```python
from build123d import *

# Parameters (mm, degrees)
EXTRUDE_1_DEPTH     = 6
SKETCH_2_W          = 12
SKETCH_2_H          = 12
CUT_EXTRUDE_1_DEPTH = 20


with BuildPart() as part:
    # 草图1 → 凸台-拉伸1 (new body)
    with BuildSketch(Plane.XY):
        with BuildLine():
            Line((3, 0), (17, 0))
            ThreePointArc((17, 0), (19.121320344, 0.878679656), (20, 3))
            ThreePointArc((20, 3), (19.121320344, 5.121320344), (17, 6))
            Line((17, 6), (3, 6))
            ThreePointArc((3, 6), (0.878679656, 5.121320344), (0, 3))
            ThreePointArc((0, 3), (0.878679656, 0.878679656), (3, 0))
        make_face()
    extrude(amount=EXTRUDE_1_DEPTH)

    # 草图2 → 切除-拉伸1 (cut)
    with BuildSketch(Plane(origin=(0, 0, 0), x_dir=(0, 0, -1), z_dir=(1, 0, 0))):
        with Locations((-3, 3)):
            Rectangle(SKETCH_2_W, SKETCH_2_H)
        Polygon((-6, 5.7), (-6, 0.3), (-5.7, 0), (-0.3, 0), (0, 0.3), (0, 5.7), (-0.3, 6), (-5.7, 6), align=None, mode=Mode.SUBTRACT)
    extrude(amount=CUT_EXTRUDE_1_DEPTH, mode=Mode.SUBTRACT)


solid = part.part
```
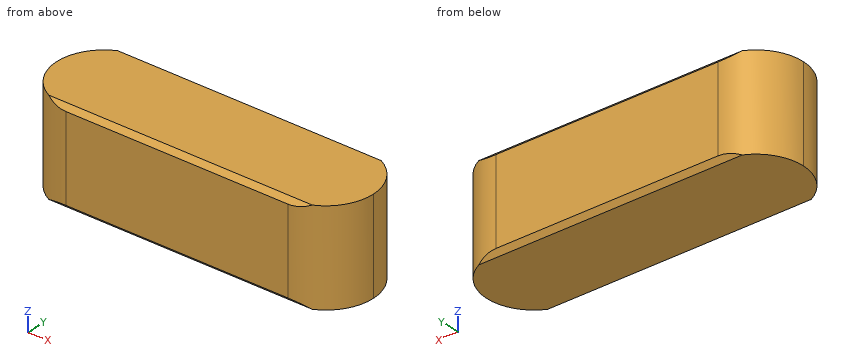
Geometry: final body of the model. Coordinates: model frame, mm. Coordinates: 2 decimals unless noted, no trailing zeros. Order: outer loops, then holes, each group sorted by start corner. A loop starts at its lowest first (then second) coordinate and runs counter-clockwise, first axis right, second up. Notation, with made-up numbers: (51.5, 51) -> (88.5, 51) arc R19 ccw to (88.5, 83) -> close; hole circle Ø7 at (82.5, 51.5). An arc over 180 degrees is marked (long way). Write each question's results on one line, items separated by ' | '. Start each with the question number.
1) Cut plane D-D, the plane y = 5.5. Output: boundary loops of the cut face in (x, z), and give its area (3 significant figures).
2) Cut plane B-B, the plane x = 2.5. Output: boundary loops of the cut face in (y, z).
3) Cut plane C-C, the plane y = 4.25. Output: boundary loops of the cut face in (x, z), and give its area (3 significant figures).
4) Cut plane A-A, the plane z = 1.7. Output: boundary loops of the cut face in (x, y).
5) First-contact query: pin 1 (2 mm diameter, centred on y = 4.5, z = 0.5, fed in from -X). Flat tip, straight axial feed; report the tip coordinate or a pass-through.
6) Material intervals for line 1 along X through (y, z) = (5, 4.4); line 2 along Y through (x, z) = (1.75, 1.95); line 3 along X through (y, z) = (4, 3.95), sorted ascending.
Checks:
1) outline: (1.34, 0) -> (18.66, 0) -> (18.66, 6) -> (1.34, 6) -> close | area: 104 mm^2
2) outline: (0.04, 0.26) -> (0.3, 0) -> (5.7, 0) -> (5.96, 0.26) -> (5.96, 5.74) -> (5.7, 6) -> (0.3, 6) -> (0.04, 5.74) -> close
3) outline: (0.27, 0) -> (19.73, 0) -> (19.73, 6) -> (0.27, 6) -> close | area: 117 mm^2
4) outline: (3, 0) -> (17, 0) arc R3 ccw to (17, 6) -> (3, 6) arc R3 ccw to start
5) pin 1: x = 0.04
6) line 1: 0.76 to 19.24 | line 2: 0.27 to 5.73 | line 3: 0.17 to 19.83
